The listing builds one solid part. Answer for the finished solid, in the listing's coordinates (mm). Face numbers are marked on the shaded views. A direction names the side the tool comes from. Round coordinates to 2 decimals unless told otherwise and drop trailing zeros. Loops run counter-clockwise (first coordinate to the right, second up) from the corner with the lowest first, then second, coordinate; pieces in that order, holes last. Notation, with made-up numbers: (10.25, 76) -> (54.25, 76) arc R20 cw to (54.25, 101) -> close; hole circle Ø9 at (-8, -20). An arc over 180 degrees is marked (long way). Write each question's results on one line, items separated by ' | '. Start each with the question number.
from build123d import *

# Parameters (mm, degrees)
BOSS_EXTRUDE1_DEPTH = 2.5
SKETCH2_R           = 2
BOSS_EXTRUDE2_DEPTH = 2
SKETCH3_R           = 2.57
BOSS_EXTRUDE3_DEPTH = 2.5
BOSS_EXTRUDE3_TAPER = 13
SKETCH4_R           = 2.57
BOSS_EXTRUDE4_DEPTH = 2.5
BOSS_EXTRUDE4_TAPER = 12
SKETCH5_R           = 2.5
SKETCH5_R_2         = 1.15
BOSS_EXTRUDE5_DEPTH = 4.1
SKETCH6_R           = 1.15
CUT_EXTRUDE1_DEPTH  = 11.666370528
FILLET1_R           = 0.3
FILLET2_R           = 0.2


with BuildPart() as part:
    # Sketch1 → Boss-Extrude1 (new body)
    with BuildSketch(Plane(origin=(0, 0, 0), x_dir=(1, 0, 0), z_dir=(0, 1, 0))):
        Polygon((3.666174209, 0), (1.833087105, 3.175), (-1.833087105, 3.175), (-3.666174209, 0), (-1.833087105, -3.175), (1.833087105, -3.175), align=None)
    extrude(amount=BOSS_EXTRUDE1_DEPTH)

    # Sketch2 → Boss-Extrude2 (add)
    with BuildSketch(Plane(origin=(0, 2.5, 0), x_dir=(1, 0, 0), z_dir=(0, 1, 0))):
        with Locations(Location((0, 0, 0), (0, 0, 270))):
            Circle(SKETCH2_R)
    extrude(amount=BOSS_EXTRUDE2_DEPTH)

    # Sketch3 → Boss-Extrude3 (add)
    with BuildSketch(Plane(origin=(0, 4.5, 0), x_dir=(1, 0, 0), z_dir=(0, 1, 0))):
        Circle(SKETCH3_R)
    extrude(amount=BOSS_EXTRUDE3_DEPTH, taper=BOSS_EXTRUDE3_TAPER)

    # Sketch4 → Boss-Extrude4 (add)
    with BuildSketch(Plane(origin=(0, 7, 0), x_dir=(1, 0, 0), z_dir=(0, 1, 0))):
        Circle(SKETCH4_R)
    extrude(amount=BOSS_EXTRUDE4_DEPTH, taper=BOSS_EXTRUDE4_TAPER)

    # Sketch5 → Boss-Extrude5 (add)
    with BuildSketch(Plane.XZ):
        with Locations(Location((0, 0, 0), (0, 0, 90))):
            Circle(SKETCH5_R)
        with Locations(Location((0, 0, 0), (0, 0, 270))):
            Circle(SKETCH5_R_2, mode=Mode.SUBTRACT)
    extrude(amount=BOSS_EXTRUDE5_DEPTH)

    # Sketch6 → Cut-Extrude1 (cut, through all)
    with BuildSketch(Plane.XZ):
        with Locations(Location((0, 0, 0), (0, 0, 270))):
            Circle(SKETCH6_R)
    extrude(amount=-CUT_EXTRUDE1_DEPTH, mode=Mode.SUBTRACT)

    # Fillet1
    fillet1_edges = [part.edges().sort_by_distance(p)[0] for p in [
        (1.833087105, 1.25, 3.175),
        (-1.833087105, 1.25, 3.175),
        (-3.666174209, 1.25, 0),
        (-1.833087105, 1.25, -3.175),
        (1.833087105, 1.25, -3.175),
        (3.666174209, 1.25, 0),
    ]]
    fillet(fillet1_edges, radius=FILLET1_R)

    # Fillet2
    fillet2_edges = [part.edges().sort_by_distance(p)[0] for p in [
        (-2.038608596, 9.5, 0),
        (0, -4.1, -2.5),
    ]]
    fillet(fillet2_edges, radius=FILLET2_R)


solid = part.part
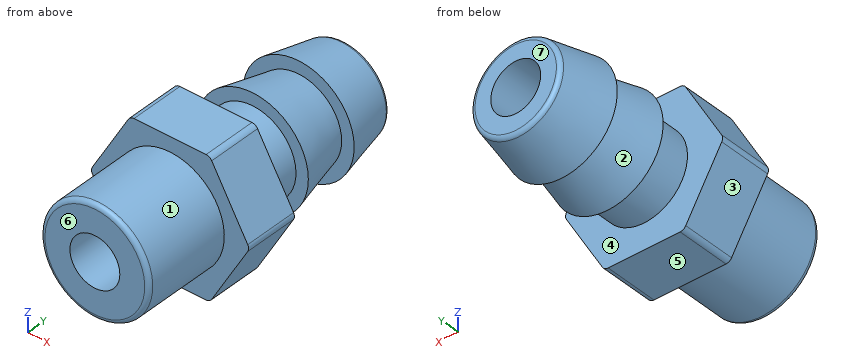
Item 1: For the marked faces 1, 2 and 3, determine the directions among +Z, -Z, +X, -X, +Y, -Y from which every point of the face is accessible in a straight line to the end or side of a thin tool.
Item 2: Straight lines are drawn through the part: L1, parallel to X at y = -1.15, z = 0; L2, parallel to X at y = 4, z = 0; L3, parallel to X at y = -2.75, z = 1.5. For each, find the intervals that lie inside material, in ascending order. Write a range as [from, to].
Item 3: The part is cut by section D-D, the plane y = 6.5. Give the vertices of the cut face in (x, z), plus the area to 3 significant figures.
Item 4: The part is cut by section B-B, the plane x = 0. Give the vertices of the cut face in (y, z) (3 decimals), plus the area to 3 significant figures.
Item 5: The part is cut by section C-C, the plane y = 8.75. Give the vertices of the cut face in (x, z).
Item 6: Each of these flat-tipped pins is pushed along its axis until it touches: pin 1 Ø1.4 at (x, z) = (0, 0) entering from +Y; pin 2 Ø2 at (y, z) = (7, 1) entering from +X; pin 3 Ø1 at (y, z) = (7, 0.5) entering from -X. Where does it stop, or does it pass through?
Item 7: The part is cut by section A-A, the plane y = 0.75. Give the vertices of the cut face in (x, z) (3 decimals).
Item 8: Determine the mould class of the marked faces 4, 5, 6 and 7 for opening direction Y: +Y half, -Y half, draft (parallel to the pull), parting line (faces both ways), or undercut.
Report:
1) face 1: -Y | face 2: none | face 3: -Z, -X, +Y, -Y
2) L1: x = [-2.5, -1.15], [1.15, 2.5] | L2: x = [-2, -1.15], [1.15, 2] | L3: x = [-2, 2]
3) outline: circle Ø4.22 at (0, 0); hole circle Ø2.3 at (0, 0) | area: 9.81 mm2
4) outline: (-4.1, -2.3) arc R0.2 ccw to (-3.9, -2.5) -> (0, -2.5) -> (0, -3.175) -> (2.5, -3.175) -> (2.5, -2) -> (4.5, -2) -> (4.5, -2.57) -> (7, -1.993) -> (7, -2.57) -> (9.342, -2.072) arc R0.2 ccw to (9.5, -1.877) -> (9.5, -1.15) -> (-4.1, -1.15) -> close; (-4.1, 1.15) -> (9.5, 1.15) -> (9.5, 1.877) arc R0.2 ccw to (9.342, 2.072) -> (7, 2.57) -> (7, 1.993) -> (4.5, 2.57) -> (4.5, 2) -> (2.5, 2) -> (2.5, 3.175) -> (0, 3.175) -> (0, 2.5) -> (-3.9, 2.5) arc R0.2 ccw to (-4.1, 2.3) -> close | area: 36.0 mm2
5) outline: circle Ø4.4 at (0, 0); hole circle Ø2.3 at (0, 0)
6) pin 1: passes through | pin 2: stops at x = 2.57 | pin 3: stops at x = -2.57
7) outline: (-3.58, -0.15) -> (-1.92, -3.025) arc R0.3 ccw to (-1.66, -3.175) -> (1.66, -3.175) arc R0.3 ccw to (1.92, -3.025) -> (3.58, -0.15) arc R0.3 ccw to (3.58, 0.15) -> (1.92, 3.025) arc R0.3 ccw to (1.66, 3.175) -> (-1.66, 3.175) arc R0.3 ccw to (-1.92, 3.025) -> (-3.58, 0.15) arc R0.3 ccw to start; hole circle Ø2.3 at (0, 0)
8) face 4: undercut | face 5: draft | face 6: -Y half | face 7: +Y half
